from build123d import *

# Parameters (mm, degrees)
SIDE_PLATE_DEPTH           = 10
MOUNTING_BLOCK_SKETCH_W    = 30
MOUNTING_BLOCK_SKETCH_H    = 50
MOUNTING_BLOCK_DEPTH       = 10
SECOND_START               = -10
SECOND_SIDE_PLATE_DEPTH    = 10
TOP_START                  = -4
TOP_RECESS_4MM_DEPTH       = 4
SIDE_RECESS_4MM_DEPTH      = 4
CROSS_HOLE_SKETCH_R        = 11
CROSS_HOLE_DEPTH           = 40
SPOT_FACE_SKETCH_R         = 15
SPOT_FACE_2MM_DEPTH        = 2
SMALL_HOLE_SKETCH_R        = 10
SMALL_HOLE_15MM_DEEP_DEPTH = 15
PIN_HOLE_SKETCH_R          = 2.5
PIN_HOLE_DEPTH             = 40


with BuildPart() as part:
    # Side Plate Sketch → Side Plate (new body)
    with BuildSketch(Plane.XY):
        with BuildLine():
            Line((0, 0), (0, -50))
            Line((0, -50), (61.578947368, -50))
            Line((61.578947368, -50), (77.289275323, -50))
            Line((77.289275323, -50), (81.583123952, -50))
            ThreePointArc((81.583123952, -50), (95, -25), (81.583123952, 0))
            Line((81.583123952, 0), (77.289275323, 0))
            Line((77.289275323, 0), (61.578947368, 0))
            Line((61.578947368, 0), (0, 0))
        make_face()
    extrude(amount=SIDE_PLATE_DEPTH)

    # Mounting Block Sketch → Mounting Block (add)
    with BuildSketch(Plane.ZY):
        with Locations((25, -25)):
            Rectangle(MOUNTING_BLOCK_SKETCH_W, MOUNTING_BLOCK_SKETCH_H)
    extrude(amount=-MOUNTING_BLOCK_DEPTH)

    # Second Plate Sketch → Second Side Plate (add)
    with BuildSketch(Plane.XY.offset(40).offset(SECOND_START)):
        with BuildLine():
            Line((10, 0), (81.583123952, 0))
            ThreePointArc((81.583123952, 0), (95, -25), (81.583123952, -50))
            Line((81.583123952, -50), (10, -50))
            Line((10, -50), (10, 0))
        make_face()
    extrude(amount=SECOND_SIDE_PLATE_DEPTH)

    # Top Recess Sketch → Top Recess 4mm (cut)
    with BuildSketch(Plane.XY.offset(40).offset(TOP_START)):
        with BuildLine():
            Line((81.583123952, 0), (26, 0))
            Line((26, 0), (44.196790465, -50))
            Line((44.196790465, -50), (81.583123952, -50))
            ThreePointArc((81.583123952, -50), (95, -25), (81.583123952, 0))
        make_face()
    extrude(amount=TOP_RECESS_4MM_DEPTH, mode=Mode.SUBTRACT)

    # Side Recess Sketch → Side Recess 4mm (cut)
    with BuildSketch(Plane(origin=(0, 0, 0), x_dir=(-1, 0, 0), z_dir=(0, 0, -1))):
        with BuildLine():
            Line((-26, 0), (-44.2, -50))
            Line((-44.2, -50), (-81.583123952, -50))
            ThreePointArc((-81.583123952, -50), (-95, -25), (-81.583123952, 0))
            Line((-81.583123952, 0), (-26, 0))
        make_face()
    extrude(amount=-SIDE_RECESS_4MM_DEPTH, mode=Mode.SUBTRACT)

    # Cross Hole Sketch → Cross Hole (cut)
    with BuildSketch(Plane.XY.offset(36)):
        with Locations((65, -23.619190871)):
            Circle(CROSS_HOLE_SKETCH_R)
    extrude(amount=-CROSS_HOLE_DEPTH, mode=Mode.SUBTRACT)

    # Spot Face Sketch → Spot Face 2mm (cut)
    with BuildSketch(Plane.ZY):
        with Locations(Location((20, -25, 0), (0, 0, 270))):
            Circle(SPOT_FACE_SKETCH_R)
    extrude(amount=-SPOT_FACE_2MM_DEPTH, mode=Mode.SUBTRACT)

    # Small Hole Sketch → Small Hole 15mm Deep (cut)
    with BuildSketch(Plane.ZY.offset(-2)):
        with Locations(Location((20, -25, 0), (0, 0, 270))):
            Circle(SMALL_HOLE_SKETCH_R)
    extrude(amount=-SMALL_HOLE_15MM_DEEP_DEPTH, mode=Mode.SUBTRACT)

    # Pin Hole Sketch → Pin Hole (cut)
    with BuildSketch(Plane.XY.offset(40)):
        with Locations((25, -32.5)):
            Circle(PIN_HOLE_SKETCH_R)
    extrude(amount=-PIN_HOLE_DEPTH, mode=Mode.SUBTRACT)


solid = part.part
The model under review builds one solid part; all positions refer to its coordinate system, in mm. A direction names the side the tool comes from. Round coordinates to 2 decimals unless told otherwise and drop trailing zeros. Loops run counter-clockwise (first coordinate to the right, second up) from the corner with the lowest first, then second, coordinate; pieces in that order, holes last. Notation, with made-up numbers: M -9,30 L 18,30 A19 ccw 18,66 Z; hole C 32,80.5 d1. An arc over 180 degrees is marked long. Answer as CSV lines item,"result".
1. We need section B-B (z = 20). Give the boundary of the cut face in (x, y).
Outcome:
outline,"M 0,-50 L 10,-50 L 10,-35 L 2,-35 L 2,-40 L 0,-40 Z; M 0,-10 L 2,-10 L 2,-15 L 10,-15 L 10,0 L 0,0 Z"
2. We need section D-D (y = -9). Give the boundary of the cut face in (x, z), plus the area to 3 significant figures.
Outcome:
outline,"M 0,0 L 29.28,0 L 29.28,4 L 90.38,4 L 90.38,10 L 10,10 L 10,30 L 90.38,30 L 90.38,36 L 29.28,36 L 29.28,40 L 0,40 Z"
area,"1,520 mm2"
3. To check wall thickness, follow L1, parallel to Z at x = 29.5, y = -29; L2, parallel to Z at x = 78.5, y = -46; L3, parallel to Y at x = 5, z = 20. State the ranges of each line that lie inside material, in increasing order. Write a range as [from, to].
Outcome:
L1,"z = [0, 10], [30, 40]"
L2,"z = [4, 10], [30, 36]"
L3,"y = [-50, -35], [-15, 0]"
4. Draft analysis for pull direction X (two halves, no side actions). For faces 1 (the face through (2, -28, 10)), 2 (the face through (52, -25, 36)), 3 (the face through (56.27, -30.31, 7.04)), state which applies: pulls with the +X half, pulls with the -X half, needs draft (parallel to the pull), parting line crosses it, or undercut.
Outcome:
face 1,"pulls with the -X half"
face 2,"needs draft"
face 3,"undercut"
5. For faces 4 (the face through (52, -25, 4)), 5 (the face through (95, -25, 7)), 6 (the face through (0.986, -21.748, 5.357)), 7 (the face through (34.97, -24.65, 37.97)), 8 (the face through (52, -25, 10)), list the 3-axis set-ups (+Z, -Z, +X, -X, +Y, -Y) from which the entire face can be reached by the end or side of a thin tool; tool diameter is ignored.
Outcome:
face 4,"-Z, +X, +Y"
face 5,"+Z, -Z, +X"
face 6,"-X"
face 7,"+Z, +X, +Y"
face 8,"+X, +Y, -Y"
6. We need section A-A (x = 52). Give the boundary of the cut face in (y, z), plus the area to 3 significant figures.
Outcome:
outline,"M -50,4 L 0,4 L 0,10 L -50,10 Z; M -50,30 L 0,30 L 0,36 L -50,36 Z"
area,"600 mm2"
7. We need section C-C (x = 65). Give the boundary of the cut face in (y, z).
Outcome:
outline,"M -50,4 L -34.62,4 L -34.62,10 L -50,10 Z; M -50,30 L -34.62,30 L -34.62,36 L -50,36 Z; M -12.62,4 L 0,4 L 0,10 L -12.62,10 Z; M -12.62,30 L 0,30 L 0,36 L -12.62,36 Z"
8. Insertion check: pin 1 Ø24 at (y, z) = (-25, 20) entering from -X; pin 2 Ø6 at (y, z) = (-25.5, 28) entering from +X; pin 3 Ø6 at (y, z) = (-15.5, 23.5) entering from +X; pin 4 Ø5 at (x, y) = (82.5, -22) entering from -Z. Each pin has a flat end and moves straight along its axis. Give the tip position at first contact, or say it passes through.
Outcome:
pin 1,"stops at x = 2"
pin 2,"stops at x = 95"
pin 3,"stops at x = 10"
pin 4,"stops at z = 4"
